```python
from build123d import *

# Parameters (mm, degrees)
BRACKET_BODY_DEPTH        = 20
MOUNTING_HOLES_SKETCH_R   = 4
MOUNTING_HOLES_2X_8_DEPTH = 20
END_SLOT_SKETCH_W         = 25
END_SLOT_SKETCH_H         = 25
END_SLOT_25_WIDE_DEPTH    = 144.380867308


with BuildPart() as part:
    # Bracket Profile Sketch → Bracket Body (new, symmetric)
    with BuildSketch(Plane(origin=(0, 0, 0), x_dir=(1, 0, 0), z_dir=(0, 1, 0))):
        with BuildLine():
            Line((-1.057217315, 3.586121305), (-14.62477547, 49.607794087))
            ThreePointArc((-14.62477547, 49.607794087), (-12.487512371, 57.644964007), (-4.367320309, 59.441203064))
            Line((-4.367320309, 59.441203064), (123.70369216, 15.732001915))
            ThreePointArc((123.70369216, 15.732001915), (125.729609358, 14.426933511), (126.909739906, 12.325782415))
            Line((126.909739906, 12.325782415), (128.559739906, 6.325782415))
            ThreePointArc((128.559739906, 6.325782415), (127.715452315, 1.969233766), (123.738712942, 0))
            Line((123.738712942, 0), (104.544556544, 0))
            ThreePointArc((104.544556544, 0), (73.738712942, 13), (42.932869341, 0))
            Line((42.932869341, 0), (3.738712942, 0))
            ThreePointArc((3.738712942, 0), (0.744501316, 0.995665256), (-1.057217315, 3.586121305))
        make_face()
    extrude(amount=BRACKET_BODY_DEPTH, both=True)

    # Mounting Holes Sketch → Mounting Holes 2xØ8 (cut, symmetric)
    with BuildSketch(Plane(origin=(0, 0, 0), x_dir=(1, 0, 0), z_dir=(0, 1, 0))):
        with Locations(Location((-6.951287058, 51.87, 0), (0, 0, 270))):
            Circle(MOUNTING_HOLES_SKETCH_R)
        with Locations(Location((0.378712942, 27, 0), (0, 0, 270))):
            Circle(MOUNTING_HOLES_SKETCH_R)
    extrude(amount=MOUNTING_HOLES_2X_8_DEPTH, both=True, mode=Mode.SUBTRACT)

    # End Slot Sketch → End Slot 25 Wide (cut, through all)
    with BuildSketch(Plane.XY):
        with Locations((-2.451287058, 0)):
            Rectangle(END_SLOT_SKETCH_W, END_SLOT_SKETCH_H)
    extrude(amount=-END_SLOT_25_WIDE_DEPTH, mode=Mode.SUBTRACT)


solid = part.part
```
Source: CAD feature listing. Evaluate the final solid. Frame: model axes, mm. A direction names the side the tool comes from. Give positions to 0.01 mm unless a question says otherwise; leave off trailing zeros. Loops run counter-clockwise (first coordinate to the right, second up) from the corner with the lowest first, then second, coordinate; pieces in that order, holes last. Notation, with made-up numbers: (78, 42.5) - (89, 42.5) arc R11 cw to (89, 63.5) - close; hole circle Ø10 at (-34.75, -38). An arc over 180 degrees is marked (long way). Use CSV: the item, a comma, the result in double quotes. Start each with the question number.
1. Draft query along Y for faces 1 (the flat face through (0, 12.5, -36)), 2 (the cylindrical face through (74, 0, -13)), 3 (the flat face through (42, -20, -24)). Return one class per face: +Y half, -Y half, draft (parallel to the pull), parting line (faces both ways), or undercut.
2. Pin query (flat end, axial travel): pin 1 (12 mm diameter, centred on x = 101.5, y = 5, fed in from -Z); pin 2 (8 mm diameter, centred on y = 5.5, z = -14.5, fed in from +X); pin 3 (10 mm diameter, centred on y = 15, z = -17, fed in from +X); pin 4 (7 mm diameter, centred on x = -6.95, z = -51.87, fed in from -Y). Return the tip coordinate at first contact, or that it passes through.
3. Section A-A (z = -27). Output: boundary loops of the cut face in (x, y).
4. Section B-B (y = 4). Output: boundary loops of the cut face in (x, z), then the cut area to 3 significant figures.
5. Section C-C (z = -46). Output: boundary loops of the cut face in (x, y).
6. Reachability of faces 4 (the flat face through (10.049, 0, -27)), 5 (the flat face through (24, 0, 0)) from +Z, -Z, +X, -X, +Y, -Y: full face, straight path, thin tool, end or side. Return the list, or none.
7. Section D-D (x = 67). Output: boundary loops of the cut face in (y, z), then the cut area to 3 significant figures.
8. Ray query, L1, parallel to Y at x = -4.5, z = -24; L2, parallel to X at y = 14, z = -3; L3, parallel to Z at x = 79, y = 12. Return the intervals inside material, ascending.
Response:
1,face 1,"undercut"
1,face 2,"draft"
1,face 3,"-Y half"
2,pin 1,"z = -25.36"
2,pin 2,"x = 127.41"
2,pin 3,"x = 127"
2,pin 4,"through"
3,outline,"(-7.96, -20) - (-3.62, -20) - (-3.62, -12.5) - (-7.96, -12.5) - close; (-7.96, 12.5) - (-3.62, 12.5) - (-3.62, 20) - (-7.96, 20) - close; (4.38, -20) - (90.69, -20) - (90.69, 20) - (4.38, 20) - (4.38, 12.5) - (10.05, 12.5) - (10.05, -12.5) - (4.38, -12.5) - close"
4,outline,"(10.05, -54.52) - (123.7, -15.73) arc R5 ccw to (126.91, -12.33) - (128.56, -6.33) arc R5 ccw to (123.74, 0) - (104.54, 0) arc R43 cw to (42.93, 0) - (10.05, 0) - close"
4,area,"3,500 mm²"
5,outline,"(-13.56, -20) - (35.02, -20) - (35.02, 20) - (-13.56, 20) - (-13.56, 12.5) - (10.05, 12.5) - (10.05, -12.5) - (-13.56, -12.5) - close"
6,face 4,"+Z, -Z, -X"
6,face 5,"+Z, +X, -X, +Y, -Y"
7,outline,"(-20, -35.08) - (20, -35.08) - (20, -12.47) - (-20, -12.47) - close"
7,area,"905 mm²"
8,L1,"-20 to -12.5, 12.5 to 20"
8,L2,"-0.84 to 46.17, 101.31 to 128.32"
8,L3,"-30.99 to -12.68"
